Work out the finished part from the listing and answer in its coordinate system (mm). Coordinates: 2 decimals unless noted, no trailing zeros. Order: outer loops, then holes, each group sorted by start corner. A loop starts at its lowest first (then second) coordinate and runs counter-clockwise, first axis right, second up. Notation, with made-up numbers: (24, 63.25) -> (53, 63.25) arc R26 cw to (53, 90.25) -> close; hole circle Ø6 at (-2, -32.75). An arc over 180 degrees is marked (long way). Write item = value, one per line. Start each with the question number.
Q1. Straight lines are drawn through the part: L1, parallel to X at y = 390, z = 1.3; L2, parallel to Y at x = -282.5, z = 1.4; L3, parallel to X at y = -235, z = 1.15. For each, find the intervals that lie inside material, in ascending order. Write a range as from..to.
Q2. A flat-ended cylindrical pin translates along its axis: pin 1 (6.5 mm diameter, centred on x = 297.5, y = 390, fed in from -Z). Find the tip coordinate at first contact, or state that the pin passes through.
Q3. The part is cut by section A-A, the plane y = 227.5. Determine the outline of the cut face in (x, z).
Q4. The part is cut by section B-B, the plane z = 0.4. Count the separate pieces of the cut face and the enclosed holes in it, plus the area to 3 significant figures.
```python
from build123d import *

# Parameters (mm, degrees)
SKETCH1_W            = 615
SKETCH1_H            = 900
BOSS_EXTRUDE1_DEPTH  = 2
SKETCH7_W            = 45
SKETCH7_H            = 91
CUT_EXTRUDE4_DEPTH   = 546.03233849
SKETCH8_R            = 2.25
CUT_EXTRUDE5_DEPTH   = 546.03233849
FILLET3_R            = 10
CUT_EXTRUDE6_DEPTH   = 10
LPATTERN1_COUNT      = 3
LPATTERN1_PITCH      = 385
LPATTERN1_COUNT_DIR2 = 2
LPATTERN1_PITCH_DIR2 = 580


with BuildPart() as part:
    # Sketch1 → Boss-Extrude1 (new body)
    with BuildSketch(Plane.XY):
        Rectangle(SKETCH1_W, SKETCH1_H)
    extrude(amount=BOSS_EXTRUDE1_DEPTH)

    # Sketch7 → Cut-Extrude4 (cut, through all)
    with BuildSketch(Plane(origin=(0, 0, 0), x_dir=(-1, 0, 0), z_dir=(0, 0, -1))):
        with Locations((5, 200)):
            Rectangle(SKETCH7_W, SKETCH7_H)
        with Locations((5, -200)):
            Rectangle(SKETCH7_W, SKETCH7_H)
    extrude(amount=-CUT_EXTRUDE4_DEPTH, mode=Mode.SUBTRACT)

    # Sketch8 → Cut-Extrude5 (cut, through all)
    with BuildSketch(Plane(origin=(0, 0, 0), x_dir=(-1, 0, 0), z_dir=(0, 0, -1))):
        with Locations((5, 250)):
            Circle(SKETCH8_R)
        with Locations((5, 150)):
            Circle(SKETCH8_R)
        with Locations((5, -150)):
            Circle(SKETCH8_R)
        with Locations((5, -250)):
            Circle(SKETCH8_R)
    extrude(amount=-CUT_EXTRUDE5_DEPTH, mode=Mode.SUBTRACT)

    # Fillet3
    fillet3_edges = [part.edges().sort_by_distance(p)[0] for p in [
        (307.5, -450, 1),
        (-307.5, -450, 1),
        (-307.5, 450, 1),
        (307.5, 450, 1),
    ]]
    fillet(fillet3_edges, radius=FILLET3_R)

    # Sketch10 → Cut-Extrude6 (cut)
    with BuildSketch(Plane(origin=(0, 0, 0), x_dir=(-1, 0, 0), z_dir=(0, 0, -1))):
        with BuildLine():
            Line((292.5, 393.3), (286.9, 393.3))
            ThreePointArc((286.9, 393.3), (277, 390), (286.9, 386.7))
            Line((286.9, 386.7), (292.5, 386.7))
            ThreePointArc((292.5, 386.7), (295.8, 390), (292.5, 393.3))
        make_face()
    cut_extrude6 = extrude(amount=-CUT_EXTRUDE6_DEPTH, mode=Mode.SUBTRACT)

    # LPattern1: Cut-Extrude6 3 × 2
    with Locations(*[(j * LPATTERN1_PITCH_DIR2, -i * LPATTERN1_PITCH, 0) for i in range(LPATTERN1_COUNT) for j in range(LPATTERN1_COUNT_DIR2) if (i, j) != (0, 0)]):
        add(cut_extrude6, mode=Mode.SUBTRACT)


solid = part.part
```
Model answer:
q1.L1 = -307.5..-295.8, -277..284.2, 303..307.5
q1.L2 = -450..-385.5, -374.5..-0.5, 10.5..384.5, 395.5..450
q1.L3 = -307.5..-27.5, 17.5..307.5
q2.pin_1 = through
q3.outline = (-307.5, 0) -> (-27.5, 0) -> (-27.5, 2) -> (-307.5, 2) -> close; (17.5, 0) -> (307.5, 0) -> (307.5, 2) -> (17.5, 2) -> close
q4.separate_pieces = 1
q4.enclosed_holes = 12
q4.area = 544,000 mm2
